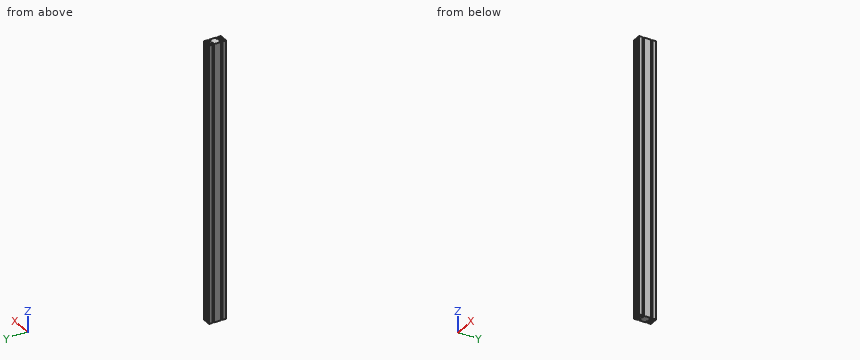
from build123d import *

# Parameters (mm, degrees)
SKETCH_1_R      = 3
EXTRUDE_1_DEPTH = 990


with BuildPart() as part:
    # 草图1 → 凸台-拉伸1 (new body)
    with BuildSketch(Plane.XY):
        Polygon((-27.495741056, 11.192504259), (-24.995741056, 11.192504259), (-24.995741056, 13.192504259), (-19.495741056, 13.192504259), (-19.495741056, 11.192504259), (-16.995741056, 11.192504259), (-16.995741056, 5.692504259), (-19.495741056, 5.692504259), (-19.495741056, 3.692504259), (-24.995741056, 3.692504259), (-24.995741056, 5.692504259), (-27.495741056, 5.692504259), (-27.495741056, -19.607495741), (-24.995741056, -19.607495741), (-24.995741056, -17.607495741), (-19.495741056, -17.607495741), (-19.495741056, -19.607495741), (-16.995741056, -19.607495741), (-16.995741056, -25.107495741), (-19.495741056, -25.107495741), (-19.495741056, -27.107495741), (-24.995741056, -27.107495741), (-24.995741056, -25.107495741), (-27.495741056, -25.107495741), (-27.495741056, -36.957495741), (-15.645741056, -36.957495741), (-15.645741056, -34.457495741), (-17.645741056, -34.457495741), (-17.645741056, -28.957495741), (-15.748076247, -28.957495741), (-15.748076247, -27.422563567), (-9.243405866, -27.422563567), (-9.243405866, -28.957495741), (-7.345741056, -28.957495741), (-7.345741056, -34.457495741), (-9.345741056, -34.457495741), (-9.345741056, -36.957495741), (2.504258944, -36.957495741), (2.504258944, -25.107495741), (0.004258944, -25.107495741), (0.004258944, -27.107495741), (-5.495741056, -27.107495741), (-5.495741056, -25.107495741), (-7.995741056, -25.107495741), (-7.995741056, -19.607495741), (-5.495741056, -19.607495741), (-5.495741056, -17.607495741), (0.004258944, -17.607495741), (0.004258944, -19.607495741), (2.504258944, -19.607495741), (2.504258944, 5.692504259), (0.004258944, 5.692504259), (0.004258944, 3.692504259), (-5.495741056, 3.692504259), (-5.495741056, 5.692504259), (-7.995741056, 5.692504259), (-7.995741056, 11.192504259), (-5.495741056, 11.192504259), (-5.495741056, 13.192504259), (0.004258944, 13.192504259), (0.004258944, 11.192504259), (2.504258944, 11.192504259), (2.504258944, 23.042504259), (-9.345741056, 23.042504259), (-9.345741056, 20.542504259), (-7.345741056, 20.542504259), (-7.345741056, 15.042504259), (-9.243405866, 15.042504259), (-9.243405866, 13.507572085), (-15.748076247, 13.507572085), (-15.748076247, 15.042504259), (-17.645741056, 15.042504259), (-17.645741056, 20.542504259), (-15.645741056, 20.542504259), (-15.645741056, 23.042504259), (-27.495741056, 23.042504259), align=None)
        with Locations((-21.995741056, 17.542504259)):
            Circle(SKETCH_1_R, mode=Mode.SUBTRACT)
        with Locations(Location((-2.995741056, 17.542504259, 0), (0, 0, 180))):
            Circle(SKETCH_1_R, mode=Mode.SUBTRACT)
        with Locations((-2.995741056, -31.457495741)):
            Circle(SKETCH_1_R, mode=Mode.SUBTRACT)
        with Locations(Location((-21.995741056, -31.457495741, 0), (0, 0, 180))):
            Circle(SKETCH_1_R, mode=Mode.SUBTRACT)
    extrude(amount=EXTRUDE_1_DEPTH)


solid = part.part
CAD build for the part. Positions are in the model's coordinates, mm. Coordinates: 2 decimals unless noted, no trailing zeros. Use one line per item in the form item = value. Start each with the question number.
1) Drill centre lines: L1, parallel to Y at x = 0.5, z = 694.5; L2, parallel to Y at x = -2.5, z = 54.5; L3, parallel to X at y = 17.5, z = 347. Where is each one in solid material? Low to high. Write a range as from..to.
2) Flat gauge pin, fed straight in: pin 1 (3 mm diameter, centred on x = -6, y = 10.5, fed in from +Z). Where does the tip first touch, or does it go through?
3) Band-saw the part on A-A (z = 885). State how many separate pieces and enclosed holes the cut face has, and give its area (3 significant figures).
Check values:
q1.L1 = -36.96..-25.11, -19.61..5.69, 11.19..23.04
q1.L2 = -36.96..-34.42, -28.5..-27.11, -17.61..3.69, 13.19..14.58, 20.5..23.04
q1.L3 = -27.5..-25, -19..-17.65, -7.35..-6, 0..2.5
q2.pin_1 = 990
q3.separate_pieces = 1
q3.enclosed_holes = 4
q3.area = 1,200 mm2
